Model file for the job. Use its own axes, mm. Face numbers are marked on the shaded views. A direction names the side the tool comes from. Coordinates: 2 decimals unless noted, no trailing zeros. Loops run counter-clockwise (first coordinate to the right, second up) from the corner with the lowest first, then second, coordinate; pieces in that order, holes last. Notation, with made-up numbers: M 47,15 L 96,15 A25 ccw 96,33 Z; hole C 13,89 d11. An arc over 180 degrees is marked long. Write item = value, one per line. Start each with the question number.
from build123d import *

# Parameters (mm, degrees)
SKETCH_1_W          = 270
SKETCH_1_H          = 30
EXTRUDE_1_DEPTH     = 40
SKETCH_2_R          = 10
CUT_EXTRUDE_2_DEPTH = 30
SKETCH_3_W          = 30
SKETCH_3_H          = 40
EXTRUDE_2_DEPTH     = 15
CUT_EXTRUDE_3_DEPTH = 159.113883008
SKETCH_5_W          = 30
SKETCH_5_H          = 40
EXTRUDE_3_DEPTH     = 15
CUT_EXTRUDE_4_DEPTH = 159.113883008


with BuildPart() as part:
    # 草图1 → 凸台-拉伸1 (new body)
    with BuildSketch(Plane(origin=(0, 0, 0), x_dir=(1, 0, 0), z_dir=(0, 1, 0))):
        Rectangle(SKETCH_1_W, SKETCH_1_H)
    extrude(amount=EXTRUDE_1_DEPTH)

    # 草图2 → 切除-拉伸2 (cut)
    with BuildSketch(Plane(origin=(0, 40, 0), x_dir=(1, 0, 0), z_dir=(0, 1, 0))):
        with Locations(Location((70, 0, 0), (0, 0, 270))):
            Circle(SKETCH_2_R)
        with Locations(Location((-70, 0, 0), (0, 0, 90))):
            Circle(SKETCH_2_R)
    extrude(amount=-CUT_EXTRUDE_2_DEPTH, mode=Mode.SUBTRACT)

    # 草图3 → 凸台-拉伸2 (add)
    with BuildSketch(Plane(origin=(135, 0, 0), x_dir=(0, 0, -1), z_dir=(1, 0, 0))):
        with Locations((0, 20)):
            Rectangle(SKETCH_3_W, SKETCH_3_H)
    extrude(amount=EXTRUDE_2_DEPTH)

    # 草图4 → 切除-拉伸3 (cut, through all)
    with BuildSketch(Plane.XY.offset(15)):
        Polygon((150, 40), (110, 0), (150, 0), align=None)
    extrude(amount=-CUT_EXTRUDE_3_DEPTH, mode=Mode.SUBTRACT)

    # 草图5 → 凸台-拉伸3 (add)
    with BuildSketch(Plane.ZY.offset(135)):
        with Locations((0, 20)):
            Rectangle(SKETCH_5_W, SKETCH_5_H)
    extrude(amount=EXTRUDE_3_DEPTH)

    # 草图6 → 切除-拉伸4 (cut, through all)
    with BuildSketch(Plane.XY.offset(15)):
        Polygon((-150, 0), (-110, 40), (-150, 40), align=None)
    extrude(amount=-CUT_EXTRUDE_4_DEPTH, mode=Mode.SUBTRACT)


solid = part.part
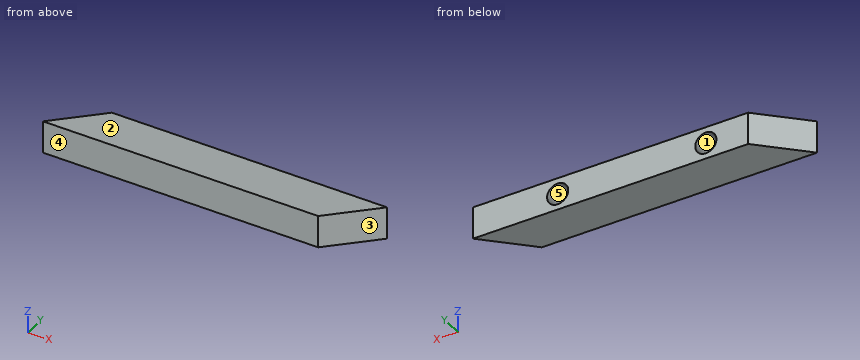
Item 1: Cut at A-A (z = 0). Give the cut face in (x, y), plus the area to 3 significant figures.
Item 2: Cut at C-C (x = -70). Give the cut face in (y, z), plus the area to 3 significant figures.
Item 3: 3-axis set-ups, long thin cutter, end or side, ignore diameter. For the marked faces 1 and 2: which of +Z, -Z, +X, -X, +Y, -Y reach the whole face in a straight line?
Item 4: Pull direction X, two halves, no side cores. Call the marked faces 3, 4 and 5: +X half, -X half, draft (parallel to the pull), parting line (faces both ways), or undercut.
Item 5: Cut at D-D (x = -114.5). Give the cut face in (y, z), plus the area to 4 significant figures.
Item 6: Pin check, flat tips, straight feed: pin 1 Ø6 at (x, z) = (69.5, 2) entering from +Y; pin 2 Ø12 at (y, z) = (33, -7.5) entering from -X; pin 3 Ø10 at (y, z) = (28, -12) entering from -X. Stop position of each tip, or through.
Item 7: Probe L1, parallel to Z at x = -70, y = 30.5; L2, parallel to X at y = 35, z = -6; L3, parallel to X at y = 24, z = 7. List the from-to ranges inside material, lowest first.
Item 8: Cut at B-B (y = 28.5). Give the cut face in (x, z).
Reported:
q1.outline = M -150,0 L 110,0 L 150,40 L 80,40 L 80,10 L 60,10 L 60,40 L -60,40 L -60,10 L -80,10 L -80,40 L -110,40 Z
q1.area = 9,200 mm^2
q2.outline = M 0,-15 L 40,-15 L 40,-10 L 10,-10 L 10,10 L 40,10 L 40,15 L 0,15 Z
q2.area = 600 mm^2
q3.face_1 = +Y
q3.face_2 = +Z, +X, -X, +Y, -Y
q4.face_3 = +X half
q4.face_4 = draft
q4.face_5 = undercut
q5.outline = M 0,-15 L 35.5,-15 L 35.5,15 L 0,15 Z
q5.area = 1,065 mm^2
q6.pin_1 = 10
q6.pin_2 = -123
q6.pin_3 = -127
q7.L1 = -15 to -10, 10 to 15
q7.L2 = -115 to -78, -62 to 62, 78 to 145
q7.L3 = -126 to -77.14, -62.86 to 62.86, 77.14 to 134
q8.outline = M -121.5,-15 L 138.5,-15 L 138.5,15 L -121.5,15 Z; hole C -70,0 d20; hole C 70,0 d20
